```python
from build123d import *

# Parameters (mm, degrees)
SKETCH1_W                                           = 48
SKETCH1_H                                           = 46
BOSS_EXTRUDE1_DEPTH                                 = 5
SKETCH2_W                                           = 38
SKETCH2_H                                           = 36
CUT_EXTRUDE1_DEPTH                                  = 35.713109915
FILLET1_R                                           = 10
CBORE_FOR_M4_HEX_SOCKET_HEAD_CAP_SCREW1_D           = 4.5
CBORE_FOR_M4_HEX_SOCKET_HEAD_CAP_SCREW1_CBORE_D     = 8
CBORE_FOR_M4_HEX_SOCKET_HEAD_CAP_SCREW1_CBORE_DEPTH = 4.4
CBORE_FOR_M4_HEX_SOCKET_HEAD_CAP_SCREW2_D           = 4.5
CBORE_FOR_M4_HEX_SOCKET_HEAD_CAP_SCREW2_CBORE_D     = 8
CBORE_FOR_M4_HEX_SOCKET_HEAD_CAP_SCREW2_CBORE_DEPTH = 4.4


with BuildPart() as part:
    # Sketch1 → Boss-Extrude1 (new, symmetric)
    with BuildSketch(Plane(origin=(0, 0, 0), x_dir=(0, 0, -1), z_dir=(1, 0, 0))):
        Rectangle(SKETCH1_W, SKETCH1_H)
    extrude(amount=BOSS_EXTRUDE1_DEPTH, both=True)

    # Sketch2 → Cut-Extrude1 (cut, through all)
    with BuildSketch(Plane(origin=(5, 0, 0), x_dir=(0, 0, -1), z_dir=(1, 0, 0))):
        with Locations((-5, 5)):
            Rectangle(SKETCH2_W, SKETCH2_H)
    extrude(amount=-CUT_EXTRUDE1_DEPTH, mode=Mode.SUBTRACT)

    # Fillet1
    fillet1_edges = [part.edges().sort_by_distance(p)[0] for p in [
        (0, -13, -14),
    ]]
    fillet(fillet1_edges, radius=FILLET1_R)

    # CBORE for M4 Hex Socket Head Cap Screw1 (through all)
    with Locations(Plane(origin=(0, -13, 0), x_dir=(1, 0, 0), z_dir=(0, 1, 0))):
        with Locations((0, -18), (0, -6)):
            CounterBoreHole(CBORE_FOR_M4_HEX_SOCKET_HEAD_CAP_SCREW1_D / 2, CBORE_FOR_M4_HEX_SOCKET_HEAD_CAP_SCREW1_CBORE_D / 2, CBORE_FOR_M4_HEX_SOCKET_HEAD_CAP_SCREW1_CBORE_DEPTH)

    # CBORE for M4 Hex Socket Head Cap Screw2 (through all)
    with Locations(Plane.XY.offset(-14)):
        with Locations((0, 17), (0, 5)):
            CounterBoreHole(CBORE_FOR_M4_HEX_SOCKET_HEAD_CAP_SCREW2_D / 2, CBORE_FOR_M4_HEX_SOCKET_HEAD_CAP_SCREW2_CBORE_D / 2, CBORE_FOR_M4_HEX_SOCKET_HEAD_CAP_SCREW2_CBORE_DEPTH)


solid = part.part
```
Input: part model. Units: mm. Frame: model coordinates. A direction names the side the tool comes from. Give positions to 0.01 mm unless a question says otherwise; leave off trailing zeros. Loops run counter-clockwise (first coordinate to the right, second up) from the corner with the lowest first, then second, coordinate; pieces in that order, holes last.
1) Contact query for flat-ended pins moving along their axis: pin 1 (4 mm diameter, centred on x = 2, z = 5, fed in from +Y); pin 2 (1 mm diameter, centred on x = 3.5, y = 1.5, fed in from +Z); pin 3 (5 mm diameter, centred on x = 0, z = 18, fed in from +Y); pin 4 (4 mm diameter, centred on x = 0, z = 6, fed in from -Y). Output: stop coordinate, or through.
A:
pin 1: stops at y = -13
pin 2: stops at z = -14
pin 3: stops at y = -17.4
pin 4: passes through
2) Line query: L1, parallel to Y at x = 0, z = -15.2; L2, parallel to Z at x = 0, y = -20.25; L3, parallel to Y at x = 0, z = -19. Output: solid intervals per line, ascending.
A:
L1: y = -23 to 1, 9 to 13, 21 to 23
L2: z = -24 to 3.75, 8.25 to 15.75, 20.25 to 24
L3: y = -23 to 2.75, 7.25 to 14.75, 19.25 to 23
3) Mould query, pull axis Z, two halves, no side actions, for faces 1 (the cylindrical face through (-0.07, -10.15, -10.99)), 2 (the cylindrical face through (-0.521, -15.169, 14.034)), 3 (the flat face through (2, -17.4, 8)), 4 (the cylindrical face through (-0.521, 20.966, -16.169)). Classes: released by +Z, released by -Z, zero draft, split by the parting line, or undercut.
A:
face 1: released by +Z
face 2: undercut
face 3: undercut
face 4: zero draft
4) Section query A-A on z = -17. Return the cut outline in (x, y).
A:
outline: (-5, -23) - (5, -23) - (5, 23) - (-5, 23) - close; hole circle Ø8 at (0, 5); hole circle Ø8 at (0, 17)
5) Reachability of faces 5 (the flat face through (0, 23, -19)), 6 (the cylindrical face through (0.488, 14.804, -21.239)), 7 (the flat face through (0, 10, -14)), 8 (the flat face through (2, 15, -18.4)), 9 (the cylindrical face through (-0.867, -15.169, 9.905)) from +Z, -Z, +X, -X, +Y, -Y: full face, straight path, thin tool, end or side. Return the list, or none.
A:
face 5: +Z, -Z, +X, -X, +Y
face 6: +Z, -Z
face 7: +Z, +X, -X, +Y
face 8: +Z
face 9: +Y
6) Section query C-C on z = 6. Return the cut outline in (x, y), and give its area (3 significant figures).
A:
outline: (-5, -23) - (-2.25, -23) - (-2.25, -17.4) - (-4, -17.4) - (-4, -13) - (-5, -13) - close; (2.25, -23) - (5, -23) - (5, -13) - (4, -13) - (4, -17.4) - (2.25, -17.4) - close
area: 39.6 mm2
7) Section query B-B on y = 5. Return the cut outline in (x, z).
A:
outline: (-5, -24) - (-2.25, -24) - (-2.25, -18.4) - (-4, -18.4) - (-4, -14) - (-5, -14) - close; (2.25, -24) - (5, -24) - (5, -14) - (4, -14) - (4, -18.4) - (2.25, -18.4) - close
8) Section query D-D on x = 0. Count the separate pieces of the cut face and the enclosed holes in it, and give its area (3 significant figures).
A:
separate pieces: 5
enclosed holes: 0
area: 620 mm2
